from build123d import *
from build123d.topology import SkipClean

# Parameters (mm, degrees)
BASE_DISC_SKETCH_R    = 32
BASE_DISC_64_DEPTH    = 3
CAGE_POSTS_6X_DEPTH   = 40
TOP_START             = -3
TOP_RING_SKETCH_R     = 32
TOP_RING_DEPTH        = 3
HUB_SKETCH_R          = 8
HUB_16_DEPTH          = 17
HUB_BORE_SKETCH_R     = 3.25
HUB_BORE_6_5_DEPTH    = 12
INNER_START           = -12
INNER_RECESS_SKETCH_R = 24
INNER_RECESS_48_DEPTH = 12


with BuildPart() as part:
    # Base Disc Sketch → Base Disc Ø64 (new body)
    with BuildSketch(Plane(origin=(0, 0, 0), x_dir=(1, 0, 0), z_dir=(0, 1, 0))):
        with Locations(Location((0, 0, 0), (0, 0, 270))):
            Circle(BASE_DISC_SKETCH_R)
    extrude(amount=BASE_DISC_64_DEPTH)

    # Cage Posts Sketch → Cage Posts 6x (add)
    with SkipClean():  # the faces are left unmerged after this step: merging them gives an invalid solid
        with BuildSketch(Plane(origin=(0, 3, 0), x_dir=(1, 0, 0), z_dir=(0, 1, 0))):
            with BuildLine():
                Line((-19.928290222, -22.734822717), (-20.828290222, -24.293668443))
                ThreePointArc((-20.828290222, -24.293668443), (-18.493333323, -26.115065051), (-16, -27.712812921))
                Line((-16, -27.712812921), (-12, -20.784609691))
                Line((-12, -20.784609691), (-13.275577673, -19.993975029))
                Line((-13.275577673, -19.993975029), (-16.125577673, -24.93031983))
                Line((-16.125577673, -24.93031983), (-19.928290222, -22.734822717))
            make_face()
            with BuildLine():
                Line((29.653079134, -5.890994228), (31.453079134, -5.890994228))
                ThreePointArc((31.453079134, -5.890994228), (31.862976417, -2.958163933), (32, 0))
                Line((32, 0), (24, 0))
                Line((24, 0), (23.953079134, -1.5))
                Line((23.953079134, -1.5), (29.653079134, -1.5))
                Line((29.653079134, -1.5), (29.653079134, -5.890994228))
            make_face()
            with BuildLine():
                ThreePointArc((20.828290222, 24.293668443), (18.493333323, 26.115065051), (16, 27.712812921))
                Line((16, 27.712812921), (12, 20.784609691))
                Line((12, 20.784609691), (13.275577673, 19.993975029))
                Line((13.275577673, 19.993975029), (16.125577673, 24.93031983))
                Line((16.125577673, 24.93031983), (19.928290222, 22.734822717))
                Line((19.928290222, 22.734822717), (20.828290222, 24.293668443))
            make_face()
            with BuildLine():
                Line((-32, 0), (-24, 0))
                ThreePointArc((-24, 0), (-23.988266915, 0.750366838), (-23.953079134, 1.5))
                Line((-23.953079134, 1.5), (-29.653079134, 1.5))
                Line((-29.653079134, 1.5), (-29.653079134, 5.890994228))
                Line((-29.653079134, 5.890994228), (-31.453079134, 5.890994228))
                ThreePointArc((-31.453079134, 5.890994228), (-31.862976417, 2.958163933), (-32, 0))
            make_face()
            with BuildLine():
                Line((9.724788912, -28.625816944), (13.527501461, -26.43031983))
                Line((13.527501461, -26.43031983), (10.677501461, -21.493975029))
                Line((10.677501461, -21.493975029), (12, -20.784609691))
                Line((12, -20.784609691), (16, -27.712812921))
                ThreePointArc((16, -27.712812921), (13.369643094, -29.073228984), (10.624788912, -30.184662671))
                Line((10.624788912, -30.184662671), (9.724788912, -28.625816944))
            make_face()
            with BuildLine():
                ThreePointArc((-16, 27.712812921), (-13.369643094, 29.073228984), (-10.624788912, 30.184662671))
                Line((-10.624788912, 30.184662671), (-9.724788912, 28.625816944))
                Line((-9.724788912, 28.625816944), (-13.527501461, 26.43031983))
                Line((-13.527501461, 26.43031983), (-10.677501461, 21.493975029))
                Line((-10.677501461, 21.493975029), (-12, 20.784609691))
                Line((-12, 20.784609691), (-16, 27.712812921))
            make_face()
        extrude(amount=CAGE_POSTS_6X_DEPTH)

    # Top Ring Sketch → Top Ring (add)
    with SkipClean():  # the faces are left unmerged after this step: merging them gives an invalid solid
        with BuildSketch(Plane(origin=(0, 43, 0), x_dir=(1, 0, 0), z_dir=(0, 1, 0)).offset(TOP_START)):
            with Locations(Location((0, 0, 0), (0, 0, 270))):
                Circle(TOP_RING_SKETCH_R)
        extrude(amount=TOP_RING_DEPTH)

    # Hub Sketch → Hub Ø16 (add)
    with SkipClean():  # the faces are left unmerged after this step: merging them gives an invalid solid
        with BuildSketch(Plane.XZ):
            with Locations(Location((0, 0, 0), (0, 0, 270))):
                Circle(HUB_SKETCH_R)
        extrude(amount=HUB_16_DEPTH)

    # Hub Bore Sketch → Hub Bore Ø6.5 (cut)
    with SkipClean():  # the faces are left unmerged after this step: merging them gives an invalid solid
        with BuildSketch(Plane.XZ.offset(17)):
            with Locations(Location((0, 0, 0), (0, 0, 270))):
                Circle(HUB_BORE_SKETCH_R)
        extrude(amount=-HUB_BORE_6_5_DEPTH, mode=Mode.SUBTRACT)

    # Inner Recess Sketch → Inner Recess Ø48 (cut)
    with SkipClean():  # the faces are left unmerged after this step: merging them gives an invalid solid
        with BuildSketch(Plane(origin=(0, 43, 0), x_dir=(1, 0, 0), z_dir=(0, 1, 0)).offset(INNER_START)):
            with Locations(Location((0, 0, 0), (0, 0, 116.416678302))):
                Circle(INNER_RECESS_SKETCH_R)
        extrude(amount=INNER_RECESS_48_DEPTH, mode=Mode.SUBTRACT)


solid = part.part
Could you check a few things on this model? Use its own coordinates, in mm. A direction names the side the tool comes from. Give positions to 0.01 mm unless a question says otherwise; leave off trailing zeros. Order: outer loops, then holes, each group sorted by start corner. A loop starts at its lowest first (then second) coordinate and runs counter-clockwise, first axis right, second up.
1. Suppose I cut it at D-D (x = -25.5). Write out the boundary of the cut face in (y, z).
Answers below:
outline: (0, -19.33) - (3, -19.33) - (3, -1.5) - (40, -1.5) - (40, -19.33) - (43, -19.33) - (43, 19.33) - (40, 19.33) - (40, 0) - (3, 0) - (3, 19.33) - (0, 19.33) - close
2. For pin 1 (4.5 mm diameter, centred on x = -27.5, y = 19, fed in from -Z); pin 2 (6 mm diameter, centred on x = 5, y = -7.5, fed in from -Z); pin 3 (5 mm diameter, centred on x = 20, y = 36.5, fed in from -Z), each with a flat end and sliding along its axis, tell me the tip position at first contact or that it passes through.
Answers below:
pin 1: stops at z = -5.89
pin 2: stops at z = -7.75
pin 3: stops at z = -26.79
3. Suppose I cut it at B-B (z = -13). Write out the boundary of the cut face in (x, y).
Answers below:
outline: (-29.24, 0) - (29.24, 0) - (29.24, 3) - (-29.24, 3) - close; (-29.24, 40) - (-20.17, 40) - (-20.17, 43) - (-29.24, 43) - close; (20.17, 40) - (29.24, 40) - (29.24, 43) - (20.17, 43) - close
4. Suppose I cut it at A-A (x = 0). Write out the boundary of the cut face in (y, z), plus the area to 3 significant figures.
Answers below:
outline: (-17, -8) - (0, -8) - (0, -32) - (3, -32) - (3, 32) - (0, 32) - (0, 8) - (-17, 8) - (-17, 3.25) - (-5, 3.25) - (-5, -3.25) - (-17, -3.25) - close; (40, -32) - (43, -32) - (43, -24) - (40, -24) - close; (40, 24) - (43, 24) - (43, 32) - (40, 32) - close
area: 434 mm2
5. Thinking about a two-plate mould opening in Z: for faces 1 (the flat face through (-28, 21, 0)), 2 (the flat face through (24, 43, 5)), 3 (the flat face through (-27, 21, -1.5)), 4 (the cylindrical face through (-1.978, -11.084, 2.579)), which applies, +Z half, -Z half, draft (parallel to the pull), parting line (faces both ways), or undercut?
Answers below:
face 1: +Z half
face 2: draft
face 3: -Z half
face 4: undercut
6. Suppose I cut it at C-C (y = 32.5). State how many separate pieces and enclosed holes the cut face has, plus the area to 3 significant figures.
Answers below:
separate pieces: 6
enclosed holes: 0
area: 128 mm2
7. I need wall thicknesses on L1, parallel to Y at x = 9.5, z = -27.5; L2, parallel to X at y = -7.25, z = 0; L3, parallel to Y at x = -8, z = -1. Which ranges of each line are inside material? Lowest first, please.
Answers below:
L1: y = 0 to 3, 40 to 43
L2: x = -8 to -3.25, 3.25 to 8
L3: y = 0 to 3
8. Which directions (+Z, -Z, +X, -X, +Y, -Y) give clear straight access to the entire face, cutting with the end or side of a thin tool? Please do faces 5 (the flat face through (11.6, 21.241, 27.543)), 6 (the flat face through (-13.97, 21.24, -24.2)), 7 (the flat face through (-31, 21, -5.891)).
Answers below:
face 5: none
face 6: -X
face 7: -Z, +X, -X
